Build history of the part. All positions in model axes, mm. Face numbers are marked on the shaded views. A direction names the side the tool comes from. Round coordinates to 2 decimals unless told otherwise and drop trailing zeros. Write each loop counter-clockwise with the first axis right and the second up, starting at its lowest first coordinate (ties: lowest second). Pieces come first, ordered by that corner, then holes. Notation, with made-up numbers: M -14.75,34 L 17.25,34 A21 ccw 17.25,42 Z; hole C 82,63.25 d11. An arc over 180 degrees is marked long. Write item = value, one per line.
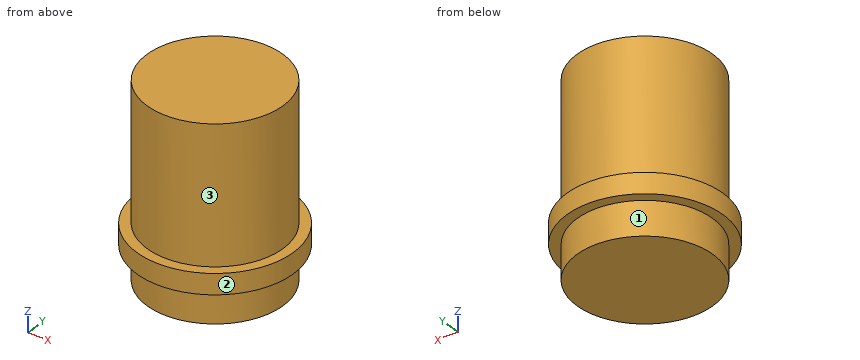
from build123d import *

# Parameters (mm, degrees)
SKETCH1_R           = 10
BOSS_EXTRUDE2_DEPTH = 5
SKETCH2_R           = 11.5
BOSS_EXTRUDE3_DEPTH = 3
SKETCH3_R           = 10
BOSS_EXTRUDE4_DEPTH = 20


with BuildPart() as part:
    # Sketch1 → Boss-Extrude2 (new body)
    with BuildSketch(Plane.XY):
        Circle(SKETCH1_R)
    extrude(amount=BOSS_EXTRUDE2_DEPTH)

    # Sketch2 → Boss-Extrude3 (add)
    with BuildSketch(Plane.XY.offset(5)):
        Circle(SKETCH2_R)
    extrude(amount=BOSS_EXTRUDE3_DEPTH)

    # Sketch3 → Boss-Extrude4 (add)
    with BuildSketch(Plane.XY.offset(8)):
        Circle(SKETCH3_R)
    extrude(amount=BOSS_EXTRUDE4_DEPTH)


solid = part.part
1. Band-saw the part on D-D (z = 5.5). List the corners of the cut face in (x, y), plus the area to 3 significant figures.
Responses:
outline = C 0,0 d23
area = 415 mm²
2. Tool access for the marked faces 1, 2 and 3: list every direction of +Z, -Z, +X, -X, +Y, -Y with a clear straight run to the whole face (end or side of a thin tool).
Responses:
face_1 = -Z
face_2 = +Z, -Z
face_3 = +Z
3. Flat gauge pins, fed straight in: pin 1 (1 mm diameter, centred on x = 2.5, y = 7.5, fed in from -Z); pin 2 (6 mm diameter, centred on x = -6.5, z = 4, fed in from +Y); pin 3 (1 mm diameter, centred on y = -5.5, z = 12, fed in from -X); pin 4 (1 mm diameter, centred on y = -1.5, z = 24.5, fed in from +X). Where does each tip first touch, or does it go through?
Responses:
pin_1 = 0
pin_2 = 10.9
pin_3 = -8.66
pin_4 = 9.95
4. Band-saw the part on C-C (z = 13.5). List the corners of the cut face in (x, y).
Responses:
outline = C 0,0 d20
5. Probe probe 1 along Z at (x, y) = (7, 8.25); probe 2 along Y at (x, z) = (0.25, 19.75); probe 3 along Y at (x, z) = (4.25, 9). List the from-to ranges inside material, lowest first.
Responses:
probe_1 = 5 to 8
probe_2 = -10 to 10
probe_3 = -9.05 to 9.05
6. Band-saw the part on A-A (x = 0). List the corners of the cut face in (y, z), plus the area to 3 significant figures.
Responses:
outline = M -11.5,5 L -10,5 L -10,0 L 10,0 L 10,5 L 11.5,5 L 11.5,8 L 10,8 L 10,28 L -10,28 L -10,8 L -11.5,8 Z
area = 569 mm²
